Can you work these out from the drawing? Everything is in mm from the part's minimum corner. A direction names the side the tool comes from. Coordinates: 2 decimals unless noted, no trailing zeros. Order: outer loops, then holes, each group sorted by start corner. A loop starts at its lowest first (then second) coordinate and runs counter-clockwise, first axis right, second up. Notation, with made-up numbers: (31.5, -3) - (68.5, -3) arc R23 cw to (68.5, 12) - close; hole circle Ø5 at (-25.75, -28). An arc over 180 degrees is marked (long way). Use a Markdown table: item, result. Add a question column.
(1) I want a section at C-C (x = 30). List the corners of the cut face in (y, z) for me.
(2) I want a section at B-B (y = 7.5). List the corners of the cut face in (x, z) for me.
(3) If I drill on L1, parallel to Y at x = 8, z = 9; L2, parallel to Y at x = 52, z = 66.5; L3, parallel to X at y = 5.25, z = 31, over which ranges is the centre line in solid material (lowest first)? Write a range as [from, to].
(4) On a 3-axis mill with a long thin cutter (end or side, diameter ignored), from which of +Z, -Z, +X, -X, +Y, -Y can I reach the whole of each face in a straight line? I mean the marked faces 4 and 5. Say none if no direction works.
(5) I want a section at D-D (z = 62.5). List the corners of the cut face in (x, y) for me.
(6) For pin 1 Ø3.5 at (x, y) = (8, 5) entering from -Z, with a flat end and sliding along its axis, tell me the tip position at first contact or that it passes through.
(7) I want a section at A-A (z = 19). List the corners of the cut face in (x, y) for me, and give its area (3 significant figures).
(8) We'd pull the mould along X, two halves only. Please class the marked faces 1, 2 and 3: pulls with the +X half, pulls with the -X half, needs draft (parallel to the pull), parting line crosses it, or undercut.
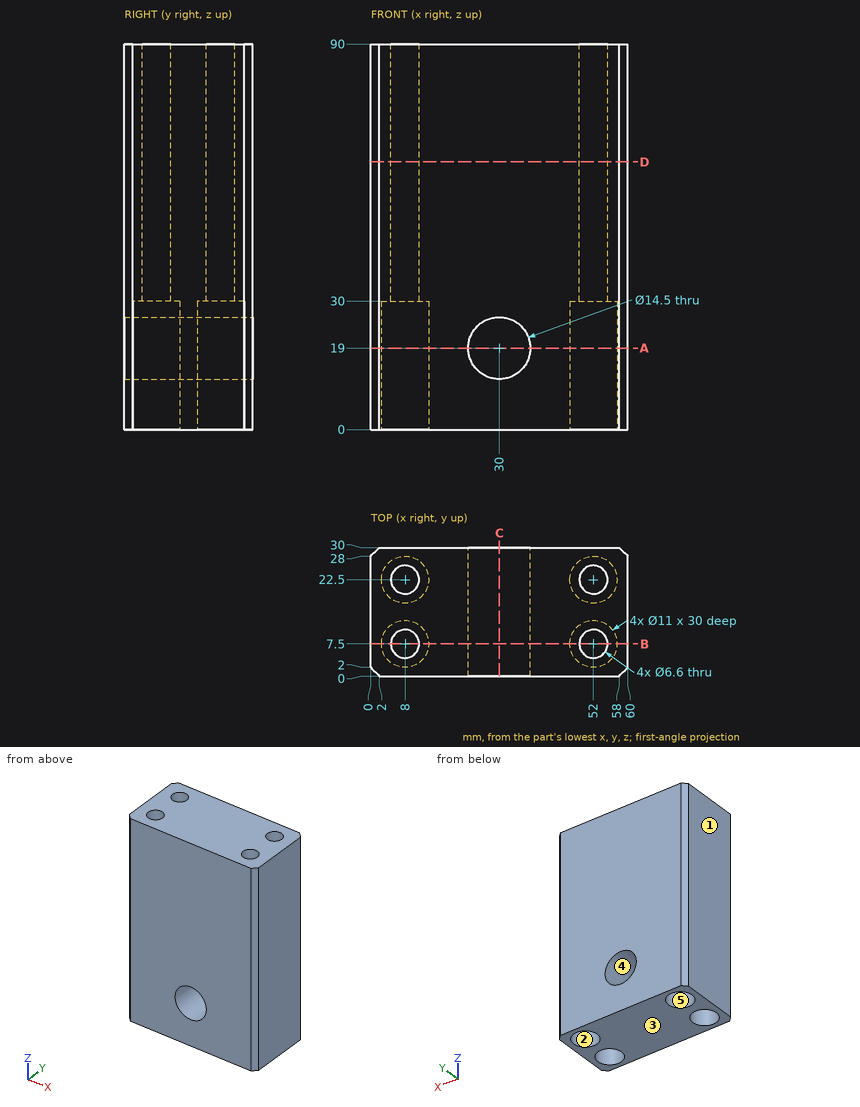
Answers follow:
| question | item | result |
|---|---|---|
| 1 | outline | (0, 0) - (30, 0) - (30, 11.75) - (0, 11.75) - close; (0, 26.25) - (30, 26.25) - (30, 90) - (0, 90) - close |
| 2 | outline | (0, 0) - (2.5, 0) - (2.5, 30) - (4.7, 30) - (4.7, 90) - (0, 90) - close; (11.3, 30) - (13.5, 30) - (13.5, 0) - (46.5, 0) - (46.5, 30) - (48.7, 30) - (48.7, 90) - (11.3, 90) - close; (55.3, 30) - (57.5, 30) - (57.5, 0) - (60, 0) - (60, 90) - (55.3, 90) - close; hole circle Ø14.5 at (30, 19) |
| 3 | L1 | y = [0, 2], [13, 17], [28, 30] |
| 3 | L2 | y = [0, 4.2], [10.8, 19.2], [25.8, 30] |
| 3 | L3 | x = [0, 5.59], [10.41, 49.59], [54.41, 60] |
| 4 | face 4 | +Y, -Y |
| 4 | face 5 | -Z |
| 5 | outline | (0, 2) - (2, 0) - (58, 0) - (60, 2) - (60, 28) - (58, 30) - (2, 30) - (0, 28) - close; hole circle Ø6.6 at (8, 7.5); hole circle Ø6.6 at (8, 22.5); hole circle Ø6.6 at (52, 7.5); hole circle Ø6.6 at (52, 22.5) |
| 6 | pin 1 | stops at z = 30 |
| 7 | outline | (0, 2) - (2, 0) - (22.75, 0) - (22.75, 30) - (2, 30) - (0, 28) - close; (37.25, 0) - (58, 0) - (60, 2) - (60, 28) - (58, 30) - (37.25, 30) - close; hole circle Ø11 at (8, 7.5); hole circle Ø11 at (8, 22.5); hole circle Ø11 at (52, 7.5); hole circle Ø11 at (52, 22.5) |
| 7 | area | 977 mm² |
| 8 | face 1 | pulls with the -X half |
| 8 | face 2 | undercut |
| 8 | face 3 | needs draft |
